Could you check a few things on this drawing? It's one solid part, dimensions in mm from its lowest x, y, z. A direction names the side the tool comes from. Give positions to 0.01 mm unless a question says otherwise; leave off trailing zeros. Order: outer loops, then holes, each group sorted by start corner. A loop starts at its lowest first (then second) coordinate and runs counter-clockwise, first axis right, second up.
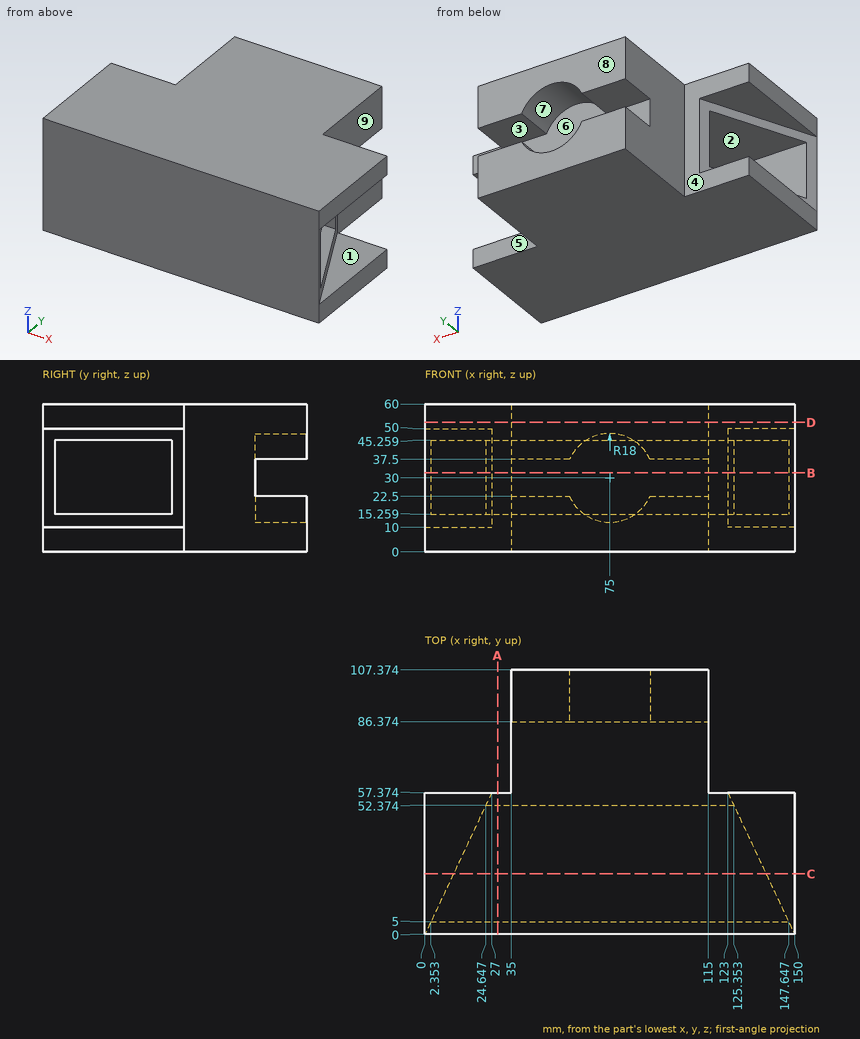
Item 1: We'd pull the mould along X, two halves only. Please class the marked faces 6, 7, 8 and 9: +X half, -X half, draft (parallel to the pull), parting line (faces both ways), or undercut.
Findings:
face 6: undercut
face 7: undercut
face 8: draft
face 9: +X half
Item 2: Imagine slicing it at A-A on x = 29.5. List the corners of the cut face in (y, z) for me, then the cut area to 3 significant figures.
Findings:
outline: (0, 0) - (57.37, 0) - (57.37, 60) - (0, 60) - close; hole (5, 15.26) - (52.37, 15.26) - (52.37, 45.26) - (5, 45.26) - close
area: 2,020 mm2
Item 3: Imagine slicing it at C-C on y = 24.5. List the corners of the cut face in (x, z) for me, then the cut area to 3 significant figures.
Findings:
outline: (0, 0) - (150, 0) - (150, 10) - (138.47, 10) - (138.47, 15.26) - (11.53, 15.26) - (11.53, 10) - (0, 10) - close; (0, 50) - (11.53, 50) - (11.53, 45.26) - (138.47, 45.26) - (138.47, 50) - (150, 50) - (150, 60) - (0, 60) - close
area: 4,270 mm2
Item 4: Imagine slicing it at B-B on z = 32. List the corners of the cut face in (x, y) for me, then the cut area to 3 significant figures.
Findings:
outline: (0, 0) - (150, 0) - (147.65, 5) - (2.35, 5) - close; (24.65, 52.37) - (125.35, 52.37) - (123, 57.37) - (115, 57.37) - (115, 86.37) - (35, 86.37) - (35, 57.37) - (27, 57.37) - close
area: 3,550 mm2
Item 5: For pin 1 (15 mm diameter, centred on y = 72.5, z = 32.5, fed in from -X); pin 2 (3 mm diameter, centred on y = 56.5, z = 26, fed in from -X); pin 3 (3 mm diameter, centred on x = 32.5, z = 21.5, fed in from +Y), each with a flat end and sliding along its axis, tell me the tip position at first contact or that it passes through.
Findings:
pin 1: stops at x = 35
pin 2: stops at x = 25.88
pin 3: stops at y = 57.37
Item 6: Imagine slicing it at D-D on z = 52.5. List the corners of the cut face in (x, y) for me.
Findings:
outline: (0, 0) - (150, 0) - (150, 57.37) - (115, 57.37) - (115, 107.37) - (35, 107.37) - (35, 57.37) - (0, 57.37) - close
Item 7: For the marked faces 1, 2, 3, 4 and 5, which set-ups out of +Z, -Z, +X, -X, +Y, -Y let a thin tool reach every point of the face, with its end or its side?
Findings:
face 1: +X, +Y
face 2: +X, -X
face 3: +X, -X, +Y
face 4: +Z, -Z, -X, +Y
face 5: +Z, -Z, +X, +Y
Item 8: Please list where these lines run through material, in increasing order: line 1 along Y through (x, z) = (49, 39.5); line 2 along Z through (x, y) = (18.5, 39); line 3 along Y through (x, z) = (99.5, 31.5).
Findings:
line 1: y = 0 to 5, 52.37 to 107.37
line 2: z = 0 to 15.26, 45.26 to 60
line 3: y = 0 to 5, 52.37 to 86.37
